Source: CAD feature listing. Evaluate the final solid. Frame: model axes, mm. A direction names the side the tool comes from. Give positions to 0.01 mm unless a question says otherwise; leave off trailing zeros. Write each loop counter-clockwise with the first axis right and the second up, starting at its lowest first coordinate (ties: lowest second). Pieces come first, ordered by that corner, then holes. Notation, with made-up numbers: M 86,-24.5 L 97,-24.5 A18 ccw 97,-13.5 Z; hole C 26,68 d4. An arc over 180 degrees is marked long. Return JSON: item names as keys, results as strings.
```python
from build123d import *

# Parameters (mm, degrees)
SKETCH1_R           = 6.5
SKETCH1_R_2         = 5.5
EXTRUDE_THIN1_DEPTH = 5
SKETCH2_W           = 6
SKETCH2_H           = 5
BOSS_EXTRUDE1_DEPTH = 3
SKETCH4_W           = 14.223079102
SKETCH4_H           = 1.5
CUT_EXTRUDE1_DEPTH  = 17.918924316


with BuildPart() as part:
    # Sketch1 → Extrude-Thin1 (new, symmetric)
    with BuildSketch(Plane.XY):
        Circle(SKETCH1_R)
        Circle(SKETCH1_R_2, mode=Mode.SUBTRACT)
    extrude(amount=EXTRUDE_THIN1_DEPTH, both=True)

    # Sketch2 → Boss-Extrude1 (add, symmetric)
    with BuildSketch(Plane.XY):
        with Locations((9, 0)):
            Rectangle(SKETCH2_W, SKETCH2_H)
    extrude(amount=BOSS_EXTRUDE1_DEPTH, both=True)

    # Sketch4 → Cut-Extrude1 (cut, through all)
    with BuildSketch(Plane.XY.offset(5)):
        with Locations((7.111539551, 0)):
            Rectangle(SKETCH4_W, SKETCH4_H)
    extrude(amount=-CUT_EXTRUDE1_DEPTH, mode=Mode.SUBTRACT)


solid = part.part
```
1) Set-up query: faces 4 (the face through (9, 2.5, 0)), 5 (the face through (-5.33, -1.9, -5)), 6 (the face through (9, 0.75, 0)). Return all of +Z, -Z, +X, -X, +Y, -Y with unobstructed straight access to the full face (end or side cutting, diameter ignored); none if empty.
Numbers:
{"face 4": "+Z, -Z, +X, +Y", "face 5": "-Z, +X, -X, +Y, -Y", "face 6": "+Z, -Z, +X"}
2) Cut plane D-D, the plane x = 0. Return the cut outline in (y, z), then the cut area to 3 significant figures.
Numbers:
{"outline": "M -6.5,-5 L -5.5,-5 L -5.5,5 L -6.5,5 Z; M 5.5,-5 L 6.5,-5 L 6.5,5 L 5.5,5 Z", "area": "20.0 mm²"}
3) Cut plane C-C, the plane z = 0.75. Return the cut outline in (x, y).
Numbers:
{"outline": "M 5.45,-0.75 A5.5 cw long 5.45,0.75 L 12,0.75 L 12,2.5 L 6,2.5 A6.5 ccw long 6,-2.5 L 12,-2.5 L 12,-0.75 Z"}
4) Cut plane A-A, the plane x = 10.5. Return the cut outline in (y, z), then the cut area to 3 significant figures.
Numbers:
{"outline": "M -2.5,-3 L -0.75,-3 L -0.75,3 L -2.5,3 Z; M 0.75,-3 L 2.5,-3 L 2.5,3 L 0.75,3 Z", "area": "21.0 mm²"}
5) Line query: line 1 (Y direction, x = 0, z = -1); line 2 (Y direction, x = 4.25, z = 4); line 3 (X direction, y = 3.5, z = -3.25). Output: solid intervals per line, ascending. Write a range as [from, to].
Numbers:
{"line 1": "y = [-6.5, -5.5], [5.5, 6.5]", "line 2": "y = [-4.92, -3.49], [3.49, 4.92]", "line 3": "x = [-5.48, -4.24], [4.24, 5.48]"}
6) Contact query for flat-ended pins moving along their axis: pin 1 Ø1.9 at (x, y) = (9, -1.5) entering from -Z; pin 2 Ø0.5 at (x, y) = (10, 2) entering from +Z; pin 3 Ø3 at (x, z) = (4, -1.5) entering from -Y. Output: stop coordinate, or through.
Numbers:
{"pin 1": "stops at z = -3", "pin 2": "stops at z = 3", "pin 3": "stops at y = -6"}
7) Cut plane B-B, the plane y = 1.25. Return the cut outline in (x, z).
Numbers:
{"outline": "M -6.38,-5 L -5.36,-5 L -5.36,5 L -6.38,5 Z; M 5.36,-5 L 6.38,-5 L 6.38,-3 L 12,-3 L 12,3 L 6.38,3 L 6.38,5 L 5.36,5 Z"}
8) Draft query along Y for faces 1 (the face through (9, -2.5, 0)), 2 (the face through (9, -0.75, 0)), 3 (the face through (12, 2, 0)). Return one class per face: released by +Y, released by -Y, zero draft, split by the parting line, or undercut.
Numbers:
{"face 1": "released by -Y", "face 2": "undercut", "face 3": "zero draft"}
